from build123d import *
from OCP.BRepFilletAPI import BRepFilletAPI_MakeChamfer

# Parameters (mm, degrees)
SKETCH_1_R                = 14
SKETCH_1_R_2              = 6.5
EXTRUDE_1_DEPTH           = 105
SKETCH_2_R                = 14
SKETCH_2_R_2              = 11
CUT_EXTRUDE_1_DEPTH       = 75
CUT_EXTRUDE_2_DEPTH       = 25
SKETCH_7_R                = 11
SKETCH_7_R_2              = 10
CUT_EXTRUDE_3_DEPTH       = 10
SKETCH_8_W                = 1
SKETCH_8_H                = 1.5
CHAMFER_1_SIZE            = 0.5
HOLE_WIZARD_4_0_4_1_D     = 4
HOLE_WIZARD_4_0_4_1_DEPTH = 8
HOLE_WIZARD_4_0_4_1_TIP   = 1.201721238
CHAMFER_2_SIZE            = 1
CHAMFER_2_SIZE2           = 1.732050808


with BuildPart() as part:
    # 草图1 → 凸台-拉伸1 (new body)
    with BuildSketch(Plane(origin=(0, 0, 0), x_dir=(0, 0, -1), z_dir=(1, 0, 0))):
        Circle(SKETCH_1_R)
        Circle(SKETCH_1_R_2, mode=Mode.SUBTRACT)
    extrude(amount=EXTRUDE_1_DEPTH)

    # 草图2 → 切除-拉伸1 (cut)
    with BuildSketch(Plane.ZY):
        Circle(SKETCH_2_R)
        Circle(SKETCH_2_R_2, mode=Mode.SUBTRACT)
    extrude(amount=-CUT_EXTRUDE_1_DEPTH, mode=Mode.SUBTRACT)

    # 草图4 → 切除-拉伸2 (cut, symmetric)
    with BuildSketch(Plane.XY):
        with BuildLine():
            Line((18, 2.5), (38, 2.5))
            ThreePointArc((38, 2.5), (40.5, 0), (38, -2.5))
            Line((38, -2.5), (18, -2.5))
            ThreePointArc((18, -2.5), (15.5, 0), (18, 2.5))
        make_face()
    extrude(amount=CUT_EXTRUDE_2_DEPTH, both=True, mode=Mode.SUBTRACT)

    # 草图7 → 切除-拉伸3 (cut)
    with BuildSketch(Plane.ZY):
        Circle(SKETCH_7_R)
        Circle(SKETCH_7_R_2, mode=Mode.SUBTRACT)
    extrude(amount=-CUT_EXTRUDE_3_DEPTH, mode=Mode.SUBTRACT)

    # 草图8 → 切除-旋转2 (revolve, cut)
    with BuildSketch(Plane.XY, mode=Mode.PRIVATE) as cut_revolve_2_sk:
        with Locations((9.5, 9.25)):
            Rectangle(SKETCH_8_W, SKETCH_8_H)
    revolve(cut_revolve_2_sk.sketch.rotate(Axis((0, 0, 0), (1, 0, 0)), 90), axis=Axis((0, 0, 0), (1, 0, 0)), mode=Mode.SUBTRACT)

    # 倒角1
    chamfer_1_edges = [part.edges().sort_by_distance(p)[0] for p in [
        (75, 0, 14),
        (105, 0, 14),
        (0, 0, -10),
    ]]
    chamfer(chamfer_1_edges, length=CHAMFER_1_SIZE)

    # Ø4.0 (4) 直径孔1
    with Locations(Plane(origin=(105, 0, 0), x_dir=(0, 0, -1), z_dir=(1, 0, 0))):
        with Locations((-10, 0), (10, 0)):
            Hole(HOLE_WIZARD_4_0_4_1_D / 2, depth=HOLE_WIZARD_4_0_4_1_DEPTH)
            with Locations((0, 0, -(HOLE_WIZARD_4_0_4_1_DEPTH + HOLE_WIZARD_4_0_4_1_TIP / 2))):  # 118° drill point
                Cone(0, HOLE_WIZARD_4_0_4_1_D / 2, HOLE_WIZARD_4_0_4_1_TIP, mode=Mode.SUBTRACT)

    # 倒角2: one chamfer whose edges measure the first distance from different faces: ONE call of the kernel's chamfer builder (chamfer() names one face for all edges)
    chamfer_2_edges_1 = [part.edges().sort_by_distance(p)[0] for p in [
        (0, 0, 6.5),
    ]]
    chamfer_2_side_1 = [part.faces().sort_by_distance(p)[0] for p in [
        (0, 0, -9.231299423),
    ]]
    chamfer_2_edges_2 = [part.edges().sort_by_distance(p)[0] for p in [
        (105, 0, 6.5),
    ]]
    chamfer_2_side_2 = [part.faces().sort_by_distance(p)[0] for p in [
        (105, 0, 13.118162338),
    ]]
    chamfer_2 = BRepFilletAPI_MakeChamfer(part.part.solid().wrapped)
    for e in chamfer_2_edges_1:
        chamfer_2.Add(CHAMFER_2_SIZE, CHAMFER_2_SIZE2, e.wrapped, chamfer_2_side_1[0].wrapped)  # the first distance lies on this face
    for e in chamfer_2_edges_2:
        chamfer_2.Add(CHAMFER_2_SIZE, CHAMFER_2_SIZE2, e.wrapped, chamfer_2_side_2[0].wrapped)  # the first distance lies on this face
    add(Compound.cast(chamfer_2.Shape()), mode=Mode.REPLACE)


solid = part.part
Part model, mm, in its own coordinate system. A direction names the side the tool comes from. Coordinates: 2 decimals unless noted, no trailing zeros. Order: outer loops, then holes, each group sorted by start corner. A loop starts at its lowest first (then second) coordinate and runs counter-clockwise, first axis right, second up. Notation, with made-up numbers: M 25.5,35.5 L 52.5,35.5 A7 cw 52.5,44.5 Z; hole C 75.5,67.5 d7. An arc over 180 degrees is marked long. Use a Markdown table: item, result.
(1) Pull direction Y, two halves, no side cores. Call faces 1 (the cylindrical face through (40.5, 0.1, -8.5)), 2 (the cylindrical face through (9.507, -8.428, -1.107)), 3 (the flat face through (75, -10, -5)): released by +Y, released by -Y, zero draft, split by the parting line, or undercut.
A:
| item | result |
|---|---|
| face 1 | undercut |
| face 2 | split by the parting line |
| face 3 | zero draft |
(2) Cut at A-A on x = 25. Write the cut outline in (y, z).
A:
| item | result |
|---|---|
| outline | M -2.5,-10.71 L -2.5,-6 A6.5 cw -2.5,6 L -2.5,10.71 A11 ccw Z; M 2.5,-10.71 A11 ccw 2.5,10.71 L 2.5,6 A6.5 cw 2.5,-6 Z |
(3) Tool access for faces 4 (the cylindrical face through (100.9, -1.2, -11.6)), 5 (the flat face through (105, -6, -6)), 6 (the cylindrical face through (15.5, -0.1, -8.5)), 7 (the flat face through (10, -8.1, 3.2)): list every direction of +Z, -Z, +X, -X, +Y, -Y with a clear straight run to the whole face (end or side of a thin tool).
A:
| item | result |
|---|---|
| face 4 | +X |
| face 5 | +Z, -Z, +X, +Y, -Y |
| face 6 | +Z, -Z |
| face 7 | none |
(4) Flat gauge pins, fed straight in: pin 1 (5 mm diameter, centred on x = 26, y = 0.5, fed in from -Z); pin 2 (6.5 mm diameter, centred on y = 1.5, z = 3, fed in from -X); pin 3 (2.5 mm diameter, centred on x = 26, z = 8, fed in from -Y). Where does each tip first touch, or does it go through?
A:
| item | result |
|---|---|
| pin 1 | stops at z = -10.71 |
| pin 2 | stops at x = 1.55 |
| pin 3 | stops at y = -8.69 |
(5) Probe L1, parallel to X at y = 7.25, z = -6; L2, parallel to Y at x = 25.5, z = 0; L3, parallel to X at y = 1.5, z = -9.25. List the from-to ranges inside material, lowest first.
A:
| item | result |
|---|---|
| L1 | x = 0 to 9, 10 to 105 |
| L2 | y = -11 to -6.5, 6.5 to 11 |
| L3 | x = 0 to 9, 10 to 16, 40 to 96.81 |
(6) Cut at C-C on x = 92.5. Write the cut outline in (y, z).
A:
| item | result |
|---|---|
| outline | C 0,0 d28; hole C 0,0 d13 |
